Geometry: see drawing. Coordinates: mm, zero at the bounding-box minimum. Round coordinates to 2 decimals unless told otherwise and drop trailing zeros. Order: outer loops, then holes, each group sorted by start corner. A loop starts at its lowest first (then second) coordinate and runs counter-clockwise, first axis right, second up. Notation, with made-up numbers: (9, 84.25) -> (54, 84.25) arc R19 cw to (54, 121.25) -> close; hole circle Ø8 at (55, -10). An arc over 180 degrees is marked (long way). Write item = value, one per line. Start each with the question number.
(1) Cut plane A-A on x = 1. Return the cut outline in (y, z), then the cut area to 3 significant figures.
(2) Cut plane D-D on y = 2.5. Return the cut outline in (x, z).
(3) Cut plane B-B on y = 4. Return the cut outline in (x, z).
(4) Ray query, line 1 (Y direction, x = 1, z = 0.3); line 2 (X direction, y = 4.05, z = 0.3); line 3 (X direction, y = 2.45, z = 0.4). Return the intervals inside material, ascending.
(5) Cut plane C-C on z = 0.15. Return the cut outline in (x, y), then the cut area to 3 significant figures.
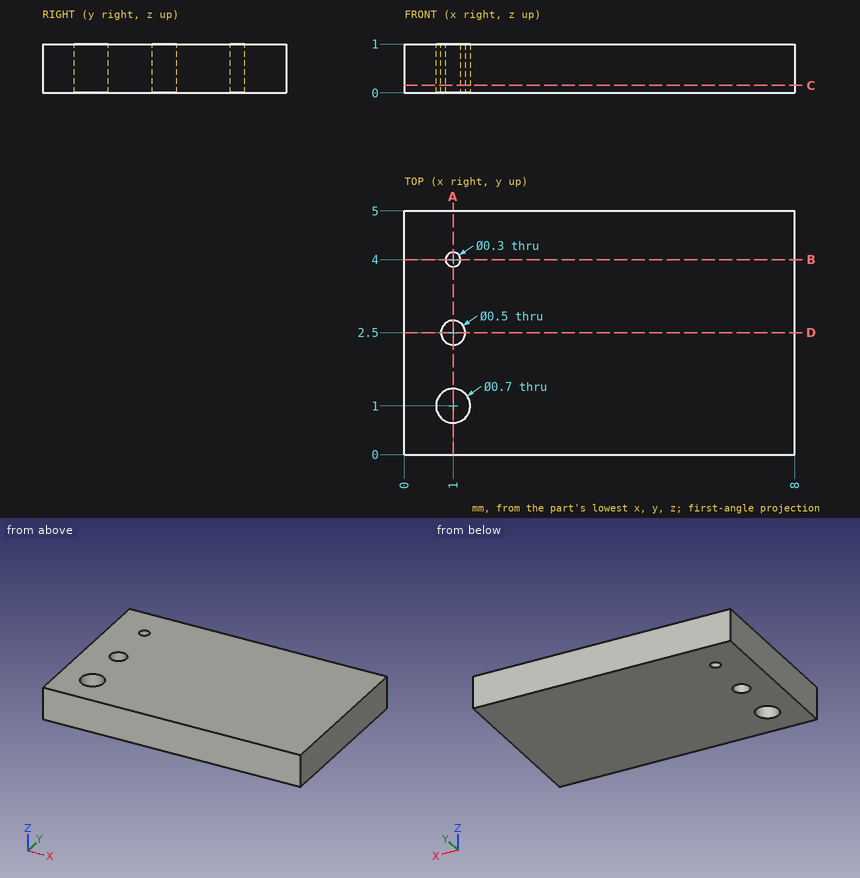
Evaluation:
q1.outline = (0, 0) -> (0.65, 0) -> (0.65, 1) -> (0, 1) -> close; (1.35, 0) -> (2.25, 0) -> (2.25, 1) -> (1.35, 1) -> close; (2.75, 0) -> (3.85, 0) -> (3.85, 1) -> (2.75, 1) -> close; (4.15, 0) -> (5, 0) -> (5, 1) -> (4.15, 1) -> close
q1.area = 3.50 mm^2
q2.outline = (0, 0) -> (0.75, 0) -> (0.75, 1) -> (0, 1) -> close; (1.25, 0) -> (8, 0) -> (8, 1) -> (1.25, 1) -> close
q3.outline = (0, 0) -> (0.85, 0) -> (0.85, 1) -> (0, 1) -> close; (1.15, 0) -> (8, 0) -> (8, 1) -> (1.15, 1) -> close
q4.line_1 = 0 to 0.65, 1.35 to 2.25, 2.75 to 3.85, 4.15 to 5
q4.line_2 = 0 to 0.86, 1.14 to 8
q4.line_3 = 0 to 0.76, 1.24 to 8
q5.outline = (0, 0) -> (8, 0) -> (8, 5) -> (0, 5) -> close; hole circle Ø0.7 at (1, 1); hole circle Ø0.5 at (1, 2.5); hole circle Ø0.3 at (1, 4)
q5.area = 39.3 mm^2
